Design review of the part built by this model. Coordinates are the model's own, in mm. A direction names the side the tool comes from. Round coordinates to 2 decimals unless told otherwise and drop trailing zeros. Loops run counter-clockwise (first coordinate to the right, second up) from the corner with the lowest first, then second, coordinate; pieces in that order, holes last. Notation, with made-up numbers: M -39,30.5 L -3,30.5 A30 ccw -3,59.5 Z; hole C 53.25,19 d3. An arc over 180 degrees is marked long. Use a Markdown table: item, result.
from build123d import *


with BuildPart() as part:
    # Sketch1 → Revolve1 (revolve)
    with BuildSketch(Plane(origin=(0, 0, 0), x_dir=(0, 0, -1), z_dir=(1, 0, 0)), mode=Mode.PRIVATE) as revolve1_sk:
        Polygon((30, 0), (30, 8), (25, 8), (25, 6), (7, 6), (7, 3), (6, 3), (6, 4), (0, 4), (0, 0), align=None)
    revolve(revolve1_sk.sketch.rotate(Axis((0, 0, 0), (0, 0, -1)), 90), axis=Axis((0, 0, 0), (0, 0, -1)))


solid = part.part
1. Take a section at A-A on y = 0. Give the boundary of the cut face in (x, z), and give its area (3 significant figures).
Check values:
| item | result |
|---|---|
| outline | M -8,-30 L 8,-30 L 8,-25 L 6,-25 L 6,-7 L 3,-7 L 3,-6 L 4,-6 L 4,0 L -4,0 L -4,-6 L -3,-6 L -3,-7 L -6,-7 L -6,-25 L -8,-25 Z |
| area | 350 mm² |
2. Wall thickness on line 1 along Z through (x, y) = (1.5, -5.25); line 2 along Z through (x, y) = (-3.75, -6.5); line 3 along X through (y, z) = (-0.25, -8.5): over which ranges is each line inside the solid? List them lowest first. Write a range as from..to.
Check values:
| item | result |
|---|---|
| line 1 | z = -30..-7 |
| line 2 | z = -30..-25 |
| line 3 | x = -5.99..5.99 |
3. Take a section at C-C on z = -5. Give the boundary of the cut face in (x, y), and give its area (3 significant figures).
Check values:
| item | result |
|---|---|
| outline | C 0,0 d8 |
| area | 50.3 mm² |
4. Insertion check: pin 1 (6 mm diameter, centred on y = -6, z = -11, fed in from -X); pin 2 (8 mm diameter, centred on y = 5, z = -6, fed in from -X); pin 3 (1.5 mm diameter, centred on y = -0.5, z = -7, fed in from +X). Each pin has a flat end and moves straight along its axis. Give the tip position at first contact, or say it passes through.
Check values:
| item | result |
|---|---|
| pin 1 | stops at x = -5.2 |
| pin 2 | stops at x = -5.89 |
| pin 3 | stops at x = 6 |
5. The part is to be moulded in two halves that separate along Z. For faces 1 (the face through (-3, 1, -7)), 2 (the face through (-2, -6, -25)), 3 (the face through (-0.867, 3.905, -2.958)), 4 (the face through (0, 0, -30)), say which applies: pulls with the +Z half, pulls with the -Z half, needs draft (parallel to the pull), parting line crosses it, or undercut.
Check values:
| item | result |
|---|---|
| face 1 | undercut |
| face 2 | pulls with the +Z half |
| face 3 | needs draft |
| face 4 | pulls with the -Z half |
6. Machinability: for faces 5 (the face through (2.86, -0.9, -6.49)), 6 (the face through (-1.73, 7.81, -27.46)), 7 (the face through (5.723, -1.802, -15.874)), which of the approach directions +Z, -Z, +X, -X, +Y, -Y give a long, thin tool a straight path to every point of the face, cutting with its end or side? Answer none if there is none.
Check values:
| item | result |
|---|---|
| face 5 | none |
| face 6 | +Z, -Z |
| face 7 | +Z |
7. Take a section at D-D on x = -5.25. Give the boundary of the cut face in (y, z), and give its area (3 significant figures).
Check values:
| item | result |
|---|---|
| outline | M -6.04,-30 L 6.04,-30 L 6.04,-25 L 2.9,-25 L 2.9,-7 L -2.9,-7 L -2.9,-25 L -6.04,-25 Z |
| area | 165 mm² |
